```python
from build123d import *

# Parameters (mm, degrees)
BOSS_EXTRUDE1_DEPTH        = 20
SKETCH2_R                  = 15
CUT_EXTRUDE1_DEPTH         = 20
M8_TAPPED_HOLE1_D          = 6.8
M8_TAPPED_HOLE1_DEPTH      = 15
M8_TAPPED_HOLE1_TIP        = 2.042926105
CHAMFER2_SIZE              = 1
SIZE_MM_DOWEL_HOLE_1_D     = 3
SIZE_MM_DOWEL_HOLE_1_DEPTH = 19.75
SIZE_MM_DOWEL_HOLE_1_TIP   = 0.901290929


with BuildPart() as part:
    # Sketch1 → Boss-Extrude1 (new body)
    with BuildSketch(Plane.XY):
        Polygon((12.5, 27), (24.5, 15), (24.5, -15), (12.5, -27), (-24.5, -27), (-24.5, 27), align=None)
    extrude(amount=BOSS_EXTRUDE1_DEPTH)

    # Sketch2 → Cut-Extrude1 (cut)
    with BuildSketch(Plane.XY.offset(20)):
        with Locations((-0.5, 0)):
            Circle(SKETCH2_R)
    extrude(amount=-CUT_EXTRUDE1_DEPTH, mode=Mode.SUBTRACT)

    # M8 Tapped Hole1
    with Locations(Plane(origin=(-0.5, 27, 10), x_dir=(0, 0, 1), z_dir=(0, 1, 0))):
        with Locations((0, 0)):
            Hole(M8_TAPPED_HOLE1_D / 2, depth=M8_TAPPED_HOLE1_DEPTH)
            with Locations((0, 0, -(M8_TAPPED_HOLE1_DEPTH + M8_TAPPED_HOLE1_TIP / 2))):  # 118° drill point
                Cone(0, M8_TAPPED_HOLE1_D / 2, M8_TAPPED_HOLE1_TIP, mode=Mode.SUBTRACT)

    # Chamfer2
    chamfer2_edges = [part.edges().sort_by_distance(p)[0] for p in [
        (-15.5, 0, 0),
        (-15.5, 0, 20),
    ]]
    chamfer(chamfer2_edges, length=CHAMFER2_SIZE)

    # Size mm dowel hole 1
    with Locations(Plane(origin=(-24.5, 0, 10), x_dir=(0, -1, 0), z_dir=(-1, 0, 0))):
        with Locations((0, 0)):
            Hole(SIZE_MM_DOWEL_HOLE_1_D / 2, depth=SIZE_MM_DOWEL_HOLE_1_DEPTH)
            with Locations((0, 0, -(SIZE_MM_DOWEL_HOLE_1_DEPTH + SIZE_MM_DOWEL_HOLE_1_TIP / 2))):  # 118° drill point
                Cone(0, SIZE_MM_DOWEL_HOLE_1_D / 2, SIZE_MM_DOWEL_HOLE_1_TIP, mode=Mode.SUBTRACT)


solid = part.part
```
Check sheet for the modelled part. Datum: model origin and axes. Units: mm. Round coordinates to 2 decimals unless told otherwise and drop trailing zeros. Order: outer loops, then holes, each group sorted by start corner. A loop starts at its lowest first (then second) coordinate and runs counter-clockwise, first axis right, second up. Notation, with made-up numbers: (17.5, 57.25) - (40.5, 57.25) arc R22 ccw to (40.5, 77.25) - close; hole circle Ø4 at (14, 8). An arc over 180 degrees is marked (long way). Write item = value, one per line.
Q1. Thickness scan on line 1 along X through (y, z) = (0, 14.75); line 2 along Y through (x, z) = (-21.5, 10); line 3 along Y through (x, z) = (-0.5, 14.25). Record the ranges inside material, lowest first.
Computed:
line_1 = -24.5 to -15.5, 14.5 to 24.5
line_2 = -27 to -1.5, 1.5 to 27
line_3 = -27 to -15, 15 to 27
Q2. Draft check along X on faces 1 (the face through (6.42, -13.31, 10.13)), 2 (the face through (-19.898, -0.325, 8.536)), 3 (the face through (18.4, 21.1, 9.9)), 4 (the face through (-1.8, 20.71, 6.86)). Enter one of: pulls with the +X half, pulls with the -X half, needs draft (parallel to the pull), parting line crosses it, or undercut.
Computed:
face_1 = undercut
face_2 = needs draft
face_3 = pulls with the +X half
face_4 = undercut
Q3. Section check D-D (z = 17). Record the boundary of the cut face in (x, y).
Computed:
outline = (-24.5, -27) - (12.5, -27) - (24.5, -15) - (24.5, 15) - (12.5, 27) - (-24.5, 27) - close; hole circle Ø30 at (-0.5, 0)
Q4. Section check C-C (z = 10). Record the boundary of the cut face in (x, y).
Computed:
outline = (-24.5, -27) - (12.5, -27) - (24.5, -15) - (24.5, 15) - (12.5, 27) - (2.9, 27) - (2.9, 14.61) arc R15 cw (long way) to (-15.42, -1.5) - (-24.5, -1.5) - close; (-24.5, 1.5) - (-15.42, 1.5) arc R15 cw to (-3.9, 14.61) - (-3.9, 27) - (-24.5, 27) - close
Q5. Go/stop test with flat-tipped pins: pin 1 (5 mm diameter, centred on x = -4.5, y = 10, fed in from -Z); pin 2 (12 mm diameter, centred on x = 17.5, z = 9.5, fed in from -Y); pin 3 (12 mm diameter, centred on x = 19.5, z = 8.5, fed in from -Y). Record where each tip stops, or that it passes through.
Computed:
pin_1 = through
pin_2 = -27
pin_3 = -26
Q6. Section check A-A (x = -0.5). Record the boundary of the cut face in (y, z), and give its area (3 significant figures).
Computed:
outline = (-27, 0) - (-16, 0) - (-15, 1) - (-15, 19) - (-16, 20) - (-27, 20) - close; (15, 1) - (16, 0) - (27, 0) - (27, 6.6) - (15, 6.6) - close; (15, 13.4) - (27, 13.4) - (27, 20) - (16, 20) - (15, 19) - close
area = 396 mm^2
Q7. Section check B-B (y = 0). Record the boundary of the cut face in (x, z).
Computed:
outline = (-24.5, 0) - (-16.5, 0) - (-15.5, 1) - (-15.5, 8.5) - (-24.5, 8.5) - close; (-24.5, 11.5) - (-15.5, 11.5) - (-15.5, 19) - (-16.5, 20) - (-24.5, 20) - close; (14.5, 1) - (15.5, 0) - (24.5, 0) - (24.5, 20) - (15.5, 20) - (14.5, 19) - close
